```python
from build123d import *
from OCP.BRepFilletAPI import BRepFilletAPI_MakeChamfer

# Parameters (mm, degrees)
BOSS_EXTRUDE1_DEPTH = 16
CHAMFER1_SIZE       = 10
CHAMFER1_SIZE2      = 12.62624927
CHAMFER2_SIZE       = 8


with BuildPart() as part:
    # Sketch1 → Boss-Extrude1 (new body)
    with BuildSketch(Plane.XY):
        with BuildLine():
            Line((0, -121), (0, 121))
            Line((0, 121), (180, 155.8))
            Line((180, 155.8), (180, 144.470997586))
            ThreePointArc((180, 144.470997586), (176.937074168, 133.834479423), (168.686448136, 126.455847884))
            Line((168.686448136, 126.455847884), (93.940655591, 90.415323041))
            ThreePointArc((93.940655591, 90.415323041), (69.188777497, 68.279428426), (60, 36.369873936))
            Line((60, 36.369873936), (60, -36.269873936))
            ThreePointArc((60, -36.269873936), (69.188777497, -68.179428426), (93.940655591, -90.315323041))
            Line((93.940655591, -90.315323041), (168.686448136, -126.355847884))
            ThreePointArc((168.686448136, -126.355847884), (176.937074168, -133.734479423), (180, -144.370997586))
            Line((180, -144.370997586), (180, -155.8))
            Line((180, -155.8), (0, -121))
        make_face()
    extrude(amount=BOSS_EXTRUDE1_DEPTH)

    # Chamfer1: one chamfer whose edges measure the first distance from different faces: ONE call of the kernel's chamfer builder (chamfer() names one face for all edges)
    chamfer1_edges_1 = [part.edges().sort_by_distance(p)[0] for p in [
        (0, -121, 8),
    ]]
    chamfer1_side_1 = [part.faces().sort_by_distance(p)[0] for p in [
        (0, 0, 8),
    ]]
    chamfer1_edges_2 = [part.edges().sort_by_distance(p)[0] for p in [
        (0, 121, 8),
    ]]
    chamfer1_side_2 = [part.faces().sort_by_distance(p)[0] for p in [
        (90, 138.4, 8),
    ]]
    chamfer1 = BRepFilletAPI_MakeChamfer(part.part.solid().wrapped)
    for e in chamfer1_edges_1:
        chamfer1.Add(CHAMFER1_SIZE, CHAMFER1_SIZE2, e.wrapped, chamfer1_side_1[0].wrapped)  # the first distance lies on this face
    for e in chamfer1_edges_2:
        chamfer1.Add(CHAMFER1_SIZE, CHAMFER1_SIZE2, e.wrapped, chamfer1_side_2[0].wrapped)  # the first distance lies on this face
    add(Compound.cast(chamfer1.Shape()), mode=Mode.REPLACE)

    # Chamfer2
    chamfer2_edges = [part.edges().sort_by_distance(p)[0] for p in [
        (0, -1.313124635, 16),
        (96.198347107, -139.598347107, 16),
        (6.198347107, -117.198347107, 16),
        (4.909096102, 115.635967278, 16),
        (94.909096102, 139.349091913, 16),
    ]]
    chamfer(chamfer2_edges, length=CHAMFER2_SIZE)


solid = part.part
```
CAD build for the part. Positions are in the model's coordinates, mm. A direction names the side the tool comes from. Round coordinates to 2 decimals unless told otherwise and drop trailing zeros. Order: outer loops, then holes, each group sorted by start corner. A loop starts at its lowest first (then second) coordinate and runs counter-clockwise, first axis right, second up. Notation, with made-up numbers: (29, -13) - (34, -13) arc R33 cw to (34, 18) - close; hole circle Ø6 at (-4, 67.5). An arc over 180 degrees is marked (long way). Answer as CSV lines item,"result". Start each with the question number.
1. Saw through at D-D, the plane x = 74.5. Write the cut outline in (y, z).
2. Saw through at A-A, the plane x = 149.5. Write the cut outline in (y, z).
3. Tool access for faces 5 (the face through (98.12, -135.953, 11.944)), 6 (the face through (68.94, -67.78, 7.89)): list every direction of +Z, -Z, +X, -X, +Y, -Y with a clear straight run to the whole face (end or side of a thin tool).
4. Saw through at C-C, the plane y = 24. Write the cut outline in (x, z), and give its area (3 significant figures).
5. Saw through at B-B, the plane z = 12.75. Write the cut outline in (x, y), and give its area (3 significant figures).
6. Pull direction Y, two halves, no side cores. Call faces 1 (the face through (176.85, -133.6, 7.89)), 2 (the face through (4.84, 115.534, 3.944)), 3 (the face through (57, 2, 16)), 4 (the face through (130.79, -108.083, 7.888)): +Y half, -Y half, draft (parallel to the pull), parting line (faces both ways), or undercut.
7. Drill centre lines: L1, parallel to X at y = 4.5, z = 3.25; L2, parallel to Y at x = 104, z = 5.25; L3, parallel to Y at x = 170.5, z = 6. Where is each one in solid material? Low to high. Write a range as [from, to].
8. Pin check, flat tips, straight feed: pin 1 (5 mm diameter, centred on x = 102.5, z = 9.5, fed in from -Y); pin 2 (1 mm diameter, centred on x = 122.5, y = -119, fed in from -Z); pin 3 (5 mm diameter, centred on x = 37, z = 8, fed in from +Y). Stop position of each tip, or through.
Model answer:
1,outline,"(-135.4, 0) - (-75.38, 0) - (-75.38, 16) - (-127.26, 16) - (-135.4, 8) - close; (75.48, 0) - (135.4, 0) - (135.4, 8) - (127.26, 16) - (75.48, 16) - close"
2,outline,"(-149.9, 0) - (-117.1, 0) - (-117.1, 16) - (-141.76, 16) - (-149.9, 8) - close; (117.2, 0) - (149.9, 0) - (149.9, 8) - (141.76, 16) - (117.2, 16) - close"
3,face 5,"+Z, -X, -Y"
3,face 6,"+Z, -Z, +X"
4,outline,"(0, 0) - (60, 0) - (60, 16) - (8, 16) - (0, 8) - close"
4,area,"928 mm²"
5,outline,"(4.75, -109.03) - (14.73, -119.01) - (180, -150.96) - (180, -144.37) arc R20 ccw to (168.69, -126.36) - (93.94, -90.32) arc R60 cw to (60, -36.27) - (60, 36.37) arc R60 cw to (93.94, 90.42) - (168.69, 126.46) arc R20 ccw to (180, 144.47) - (180, 150.96) - (12.65, 118.61) - (4.75, 106.92) - close"
5,area,"22,600 mm²"
6,face 1,"undercut"
6,face 2,"+Y half"
6,face 3,"draft"
6,face 4,"undercut"
7,L1,"x = [0, 60]"
7,L2,"y = [-141.11, -95.17], [95.27, 141.11]"
7,L3,"y = [-153.96, -127.35], [127.45, 153.96]"
8,pin 1,"stops at y = -141.2"
8,pin 2,"stops at z = 0"
8,pin 3,"stops at y = 128.64"
